For this review, take the finished solid that the model builds, in its own axes (mm). A direction names the side the tool comes from. Round coordinates to 2 decimals unless told otherwise and drop trailing zeros. Write each loop counter-clockwise with the first axis right and the second up, starting at its lowest first coordinate (ties: lowest second). Pieces come first, ordered by that corner, then holes. Notation, with made-up numbers: (13.5, 84) -> (51.5, 84) arc R21 cw to (51.5, 117) -> close; hole circle Ø8 at (73, 46.5). An arc over 180 degrees is marked (long way). Answer in a Markdown table with one row per item.
from build123d import *

# Parameters (mm, degrees)
SKETCH1_R           = 1.75
BOSS_EXTRUDE1_DEPTH = 15.5
SKETCH2_R           = 4.75
BOSS_EXTRUDE2_DEPTH = 9.5
SKETCH3_R           = 6.75
BOSS_EXTRUDE3_DEPTH = 35.5
CHAMFER1_SIZE       = 1
CHAMFER1_SIZE2      = 6
FILLET1_R           = 3


with BuildPart() as part:
    # Sketch1 → Boss-Extrude1 (new body)
    with BuildSketch(Plane.XY):
        Circle(SKETCH1_R)
    extrude(amount=BOSS_EXTRUDE1_DEPTH)

    # Sketch2 → Boss-Extrude2 (add)
    with BuildSketch(Plane.XY.offset(15.5)):
        Circle(SKETCH2_R)
    extrude(amount=BOSS_EXTRUDE2_DEPTH)

    # Sketch3 → Boss-Extrude3 (add)
    with BuildSketch(Plane.XY.offset(25)):
        Circle(SKETCH3_R)
    extrude(amount=BOSS_EXTRUDE3_DEPTH)

    # Chamfer1
    chamfer1_edges = [part.edges().sort_by_distance(p)[0] for p in [
        (-6.75, 0, 25),
    ]]
    chamfer1_side = [part.faces().sort_by_distance(p)[0] for p in [
        (-6.559081169, 0, 25),
    ]]
    chamfer(chamfer1_edges, length=CHAMFER1_SIZE, length2=CHAMFER1_SIZE2, reference=chamfer1_side[0])

    # Fillet1
    fillet1_edges = [part.edges().sort_by_distance(p)[0] for p in [
        (-6.75, 0, 60.5),
    ]]
    fillet(fillet1_edges, radius=FILLET1_R)


solid = part.part
1) For faces 1 (the cylindrical face through (2.192, -4.214, 20.184)), 2 (the cylindrical face through (-1.46, -6.59, 44.06)), list the 3-axis set-ups (+Z, -Z, +X, -X, +Y, -Y) from which the entire face can be reached by the end or side of a thin tool; tool diameter is ignored.
Solved:
| item | result |
|---|---|
| face 1 | -Z |
| face 2 | +Z, -Z |
2) Consider section A-A on y = 0. State the section outline as (x, z) points.
Solved:
| item | result |
|---|---|
| outline | (-6.75, 31) -> (-5.75, 25) -> (-4.75, 25) -> (-4.75, 15.5) -> (-1.75, 15.5) -> (-1.75, 0) -> (1.75, 0) -> (1.75, 15.5) -> (4.75, 15.5) -> (4.75, 25) -> (5.75, 25) -> (6.75, 31) -> (6.75, 57.5) arc R3 ccw to (3.75, 60.5) -> (-3.75, 60.5) arc R3 ccw to (-6.75, 57.5) -> close |
3) Consider section C-C on z = 51. State the section outline as (x, y) points.
Solved:
| item | result |
|---|---|
| outline | circle Ø13.5 at (0, 0) |
4) Clearance check with flat-ended pins moving along their axes: pin 1 Ø6 at (y, z) = (0, 8.5) entering from +X; pin 2 Ø3 at (x, z) = (-2.5, 23) entering from +Y; pin 3 Ø1.5 at (y, z) = (-2, 11.5) entering from +X; pin 4 Ø4 at (y, z) = (-4, 8.5) entering from -X. State where each tip first meets the part, or that it passes through.
Solved:
| item | result |
|---|---|
| pin 1 | x = 1.75 |
| pin 2 | y = 4.64 |
| pin 3 | x = 1.22 |
| pin 4 | through |
5) Consider section D-D on z = 9. State the section outline as (x, y) points.
Solved:
| item | result |
|---|---|
| outline | circle Ø3.5 at (0, 0) |
6) For line 1 (Z direction, x = 1.75, y = -1.75); line 2 (X direction, y = -0.5, z = 25.5); line 3 (X direction, y = 4, z = 24), list the stretches that pass through material, from the lowest coordinate up. Write a range as [from, to].
Solved:
| item | result |
|---|---|
| line 1 | [15.5, 60.5] |
| line 2 | [-5.81, 5.81] |
| line 3 | [-2.56, 2.56] |
